Could you check a few things on this drawing? It's one solid part, dimensions in mm from its lowest x, y, z. Give positions to 0.01 mm unless a question says otherwise; leave off trailing zeros. Order: outer loops, then holes, each group sorted by start corner. A loop starts at its lowest first (then second) coordinate and runs counter-clockwise, first axis right, second up.
(1) Will this pin go through, and if not, where does the flat tip stop? pin 1 (9 mm diameter, centred on x = 23.5, z = 130.5, fed in from +Y).
(2) Imagine slicing it at B-B, the plane z = 130. Write out the boundary of the cut face in (x, y).
(3) If I drill on probe 1 along Z at (x, y) = (25, 2.2); probe 2 along X at (y, z) = (6.25, 20.5); probe 3 along Z at (x, y) = (18.5, 9.25), over which ranges is the centre line in solid material (lowest first)?
(4) Imagine slicing it at D-D, the plane z = 23. Write out the boundary of the cut face in (x, y).
(5) Imagine slicing it at A-A, the plane x = 25. Write out the boundary of the cut face in (y, z), then the cut area to 3 significant figures.
(6) Imagine slicing it at C-C, the plane y = 10.75. Write out the boundary of the cut face in (x, z).
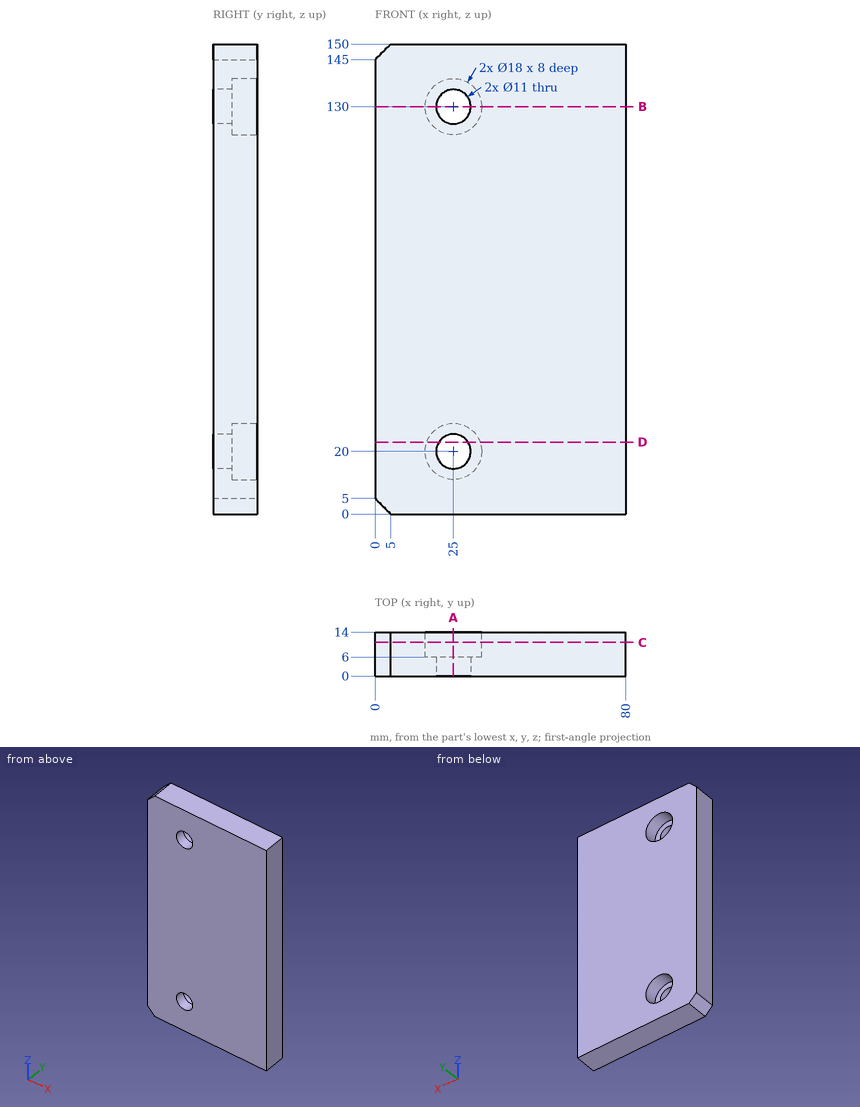
Answer block:
1. pin 1: stops at y = 6
2. outline: (0, 0) - (19.5, 0) - (19.5, 6) - (16, 6) - (16, 14) - (0, 14) - close; (30.5, 0) - (80, 0) - (80, 14) - (34, 14) - (34, 6) - (30.5, 6) - close
3. probe 1: z = 0 to 14.5, 25.5 to 124.5, 135.5 to 150
3. probe 2: x = 0 to 16.01, 33.99 to 80
3. probe 3: z = 0 to 13.78, 26.22 to 123.78, 136.22 to 150
4. outline: (0, 0) - (20.39, 0) - (20.39, 6) - (16.51, 6) - (16.51, 14) - (0, 14) - close; (29.61, 0) - (80, 0) - (80, 14) - (33.49, 14) - (33.49, 6) - (29.61, 6) - close
5. outline: (0, 0) - (14, 0) - (14, 11) - (6, 11) - (6, 14.5) - (0, 14.5) - close; (0, 25.5) - (6, 25.5) - (6, 29) - (14, 29) - (14, 121) - (6, 121) - (6, 124.5) - (0, 124.5) - close; (0, 135.5) - (6, 135.5) - (6, 139) - (14, 139) - (14, 150) - (0, 150) - close
5. area: 1,680 mm2
6. outline: (0, 5) - (5, 0) - (80, 0) - (80, 150) - (5, 150) - (0, 145) - close; hole circle Ø18 at (25, 20); hole circle Ø18 at (25, 130)
